```python
from build123d import *

# Parameters (mm, degrees)
SKETCH1_R           = 110
SKETCH1_R_2         = 90
BOSS_EXTRUDE1_DEPTH = 15
SHELL1_T            = -4


with BuildPart() as part:
    # Sketch1 → Boss-Extrude1 (new body)
    with BuildSketch(Plane.XY):
        Circle(SKETCH1_R)
        Circle(SKETCH1_R_2, mode=Mode.SUBTRACT)
    extrude(amount=BOSS_EXTRUDE1_DEPTH)

    # Shell1
    shell1_openings = [part.faces().sort_by_distance(p)[0] for p in [
        (-106.888730163, 0, 15),
    ]]
    offset(amount=SHELL1_T, openings=shell1_openings, kind=Kind.INTERSECTION)


solid = part.part
```
Verification items for the finished model (mm, model axes). A direction names the side the tool comes from. Coordinates: 2 decimals unless noted, no trailing zeros. Loops run counter-clockwise (first coordinate to the right, second up) from the corner with the lowest first, then second, coordinate; pieces in that order, holes last. Notation, with made-up numbers: (-5.5, -11) -> (-0.5, -11) arc R20 cw to (-0.5, 5) -> close; hole circle Ø1 at (35.25, 18.5). An arc over 180 degrees is marked (long way). Answer in a Markdown table with one row per item.
1) Scan lines: line 1 along Y through (x, z) = (0, 8); line 2 along X through (y, z) = (3, 9.25); line 3 along X through (y, z) = (-2, 6.5). Record each from-to range of solid material in increasing order. Write a range as from..to.
The answers:
| item | result |
|---|---|
| line 1 | y = -110..-106, -94..-90, 90..94, 106..110 |
| line 2 | x = -109.96..-105.96, -93.95..-89.95, 89.95..93.95, 105.96..109.96 |
| line 3 | x = -109.98..-105.98, -93.98..-89.98, 89.98..93.98, 105.98..109.98 |
2) Section check C-C (z = 9.5). Record the cut outline in (x, y).
The answers:
| item | result |
|---|---|
| outline | circle Ø220 at (0, 0); circle Ø188 at (0, 0); hole circle Ø212 at (0, 0); hole circle Ø180 at (0, 0) |
3) Section check A-A (y = 0). Record the cut outline in (x, z).
The answers:
| item | result |
|---|---|
| outline | (-110, 0) -> (-90, 0) -> (-90, 15) -> (-94, 15) -> (-94, 4) -> (-106, 4) -> (-106, 15) -> (-110, 15) -> close; (90, 0) -> (110, 0) -> (110, 15) -> (106, 15) -> (106, 4) -> (94, 4) -> (94, 15) -> (90, 15) -> close |
4) Draft check along Y on faces 1 (the face through (-23.846, -107.384, 7.395)), 2 (the face through (41.53, -79.845, 7.395)), 3 (the face through (-8, -94, 4)), 4 (the face through (-41, -81, 0)). Enter one of: released by +Y, released by -Y, zero draft, split by the parting line, or undercut.
The answers:
| item | result |
|---|---|
| face 1 | split by the parting line |
| face 2 | undercut |
| face 3 | undercut |
| face 4 | zero draft |
5) Depth check by flat-ended pin: P1, Ø6, axis at y = 46.5, z = 12.5, coming from the -X side; P2, Ø8, axis at x = 27.5, z = 9, coming from the +Y side; P3, Ø6, axis at x = 68.5, z = 6.5, coming from the +Y side. Enter the tip coordinate at first touch or a pass-through.
The answers:
| item | result |
|---|---|
| P1 | stops at x = -101.03 |
| P2 | stops at y = 107.46 |
| P3 | stops at y = 88.37 |
6) Access from +Z, -Z, +X, -X, +Y, -Y to the whole of each face (thin tool, end or side, straight path). Record for faces 5 (the face through (89.659, 28.235, 9.423)), 6 (the face through (76.2, -48.3, 15)).
The answers:
| item | result |
|---|---|
| face 5 | +Z |
| face 6 | +Z, +X, -X, +Y, -Y |
